Could you check a few things on this model? Use its own coordinates, in mm. Face numbers are marked on the shaded views. A direction names the side the tool comes from. Coordinates: 2 decimals unless noted, no trailing zeros. Loops run counter-clockwise (first coordinate to the right, second up) from the corner with the lowest first, then second, coordinate; pieces in that order, holes last. Notation, with made-up numbers: (59.5, 67) -> (96.5, 67) arc R7 cw to (96.5, 73) -> close; hole circle Ø3 at (89.25, 70.25). An arc over 180 degrees is marked (long way). One line per question, with ' | ' between items. Start each with the question number.
(1) I'm going to push flat-ended pins straight in: pin 1 Ø1.6 at (x, z) = (10, -1.5) entering from -Y; pin 2 Ø7.5 at (x, y) = (-5.5, 0) entering from -Z; pin 3 Ø0.6 at (x, y) = (4, -3) entering from +Z. Where does each tip first touch, or does it pass through?
(2) Suppose I cut it at A-A (z = -2). Please give me the cut outline in (x, y), plus the area to 3 significant figures.
(3) Which directions (+Z, -Z, +X, -X, +Y, -Y) give clear straight access to the entire face, cutting with the end or side of a thin tool? Please do the marked faces 1, 2 and 3.
(4) Suppose I cut it at B-B (x = -20.5). Please give me the cut outline in (y, z).
(5) If I drill on line 1 along Z through (x, y) = (3.5, -1.5); line 2 along Z through (x, y) = (4, -2.5); line 3 along X through (y, z) = (3.75, -0.75), over which ranges is the centre line in solid material (lowest first)?
```python
from build123d import *

# Parameters (mm, degrees)
SKETCH1_W           = 50
SKETCH1_H           = 25
BOSS_EXTRUDE1_DEPTH = 4
CHAMFER1_SIZE       = 4
CHAMFER1_SIZE2      = 2.309401077
SKETCH2_W           = 10
SKETCH2_H           = 10
BOSS_EXTRUDE2_DEPTH = 5.5
SKETCH3_W           = 0.8
SKETCH3_H           = 0.8
CUT_EXTRUDE1_DEPTH  = 36.780581326
LPATTERN1_COUNT     = 16
LPATTERN1_PITCH     = 2
CHAMFER2_SIZE       = 1
CHAMFER2_SIZE2      = 0.577350269


with BuildPart() as part:
    # Sketch1 → Boss-Extrude1 (new body)
    with BuildSketch(Plane.XY):
        Rectangle(SKETCH1_W, SKETCH1_H)
    extrude(amount=BOSS_EXTRUDE1_DEPTH)

    # Chamfer1
    chamfer1_edges = [part.edges().sort_by_distance(p)[0] for p in [
        (25, 0, 0),
    ]]
    chamfer1_side = [part.faces().sort_by_distance(p)[0] for p in [
        (0, 0, 0),
    ]]
    chamfer(chamfer1_edges, length=CHAMFER1_SIZE, length2=CHAMFER1_SIZE2, reference=chamfer1_side[0])

    # Sketch2 → Boss-Extrude2 (add)
    with BuildSketch(Plane(origin=(0, 0, 0), x_dir=(-1, 0, 0), z_dir=(0, 0, -1))):
        with Locations((-10, 0)):
            Rectangle(SKETCH2_W, SKETCH2_H)
    extrude(amount=BOSS_EXTRUDE2_DEPTH)

    # Sketch3 → Cut-Extrude1 (cut, through all)
    with BuildSketch(Plane(origin=(0, 12.5, 0), x_dir=(1, 0, 0), z_dir=(0, 1, 0))):
        with Locations((24, -4)):
            Rectangle(SKETCH3_W, SKETCH3_H)
    cut_extrude1 = extrude(amount=-CUT_EXTRUDE1_DEPTH, mode=Mode.SUBTRACT)

    # LPattern1: Cut-Extrude1 ×16
    with Locations(*[(-i * LPATTERN1_PITCH, 0, 0) for i in range(1, LPATTERN1_COUNT)]):
        add(cut_extrude1, mode=Mode.SUBTRACT)

    # Chamfer2
    chamfer2_edges = [part.edges().sort_by_distance(p)[0] for p in [
        (-25, 0, 0),
    ]]
    chamfer2_side = [part.faces().sort_by_distance(p)[0] for p in [
        (-3.142857143, 0, 0),
    ]]
    chamfer(chamfer2_edges, length=CHAMFER2_SIZE, length2=CHAMFER2_SIZE2, reference=chamfer2_side[0])


solid = part.part
```
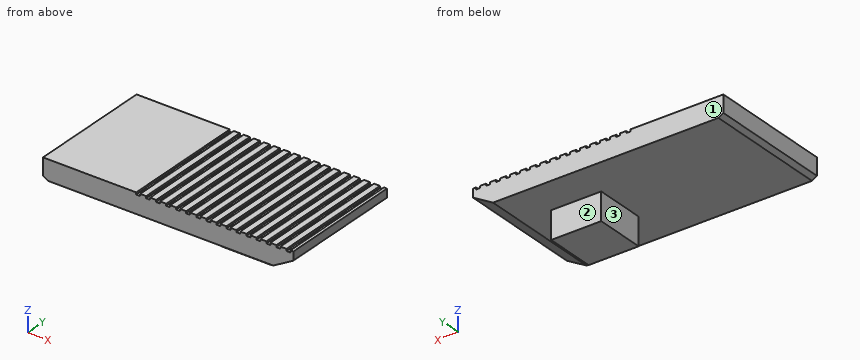
Checks:
1) pin 1: stops at y = -5 | pin 2: stops at z = 0 | pin 3: stops at z = 3.6
2) outline: (5, -5) -> (15, -5) -> (15, 5) -> (5, 5) -> close | area: 100 mm^2
3) face 1: +Z, -Z, +X, -X, +Y | face 2: -Z, +X, -X, +Y | face 3: -Z, -X, +Y, -Y
4) outline: (-12.5, 0) -> (12.5, 0) -> (12.5, 4) -> (-12.5, 4) -> close
5) line 1: z = 0 to 4 | line 2: z = 0 to 3.6 | line 3: x = 5 to 15
